```python
from build123d import *

# Parameters (mm, degrees)
SKETCH_1_W          = 350
SKETCH_1_H          = 140
EXTRUDE_1_DEPTH     = 1.5
SKETCH_2_W          = 220
SKETCH_2_H          = 110
CUT_EXTRUDE_1_DEPTH = 2
EXTRUDE_1_2_DEPTH   = 15
SKETCH_4_W          = 221.5
SKETCH_4_H          = 1.5
EXTRUDE_3_DEPTH     = 100
FILLET_1_R          = 10
CUT_EXTRUDE_2_DEPTH = 100


with BuildPart() as part:
    # 草图1 → Extrude 1 (new body)
    with BuildSketch(Plane.XY):
        Rectangle(SKETCH_1_W, SKETCH_1_H)
    extrude(amount=EXTRUDE_1_DEPTH)

    # 草图2 → 切除-拉伸1 (cut)
    with BuildSketch(Plane.XY.offset(1.5)):
        with Locations((65, 15)):
            Rectangle(SKETCH_2_W, SKETCH_2_H)
    extrude(amount=-CUT_EXTRUDE_1_DEPTH, mode=Mode.SUBTRACT)

    # 草图3 → Extrude 1 2 (add)
    with BuildSketch(Plane.XY.offset(1.5)):
        Polygon((175, -40), (175, -70), (-175, -70), (-175, 70), (-45, 70), (-45, -40), (-46.5, -40), (-46.5, 68.5), (-173.5, 68.5), (-173.5, -68.5), (173.5, -68.5), (173.5, -40), align=None)
    extrude(amount=EXTRUDE_1_2_DEPTH)

    # 草图4 → 凸台-拉伸3 (add)
    with BuildSketch(Plane.XY.offset(1.5)):
        with Locations((64.25, -40.75)):
            Rectangle(SKETCH_4_W, SKETCH_4_H)
    extrude(amount=EXTRUDE_3_DEPTH)

    # 圆角1
    fillet_1_edges = [part.edges().sort_by_distance(p)[0] for p in [
        (-46.5, -40.75, 101.5),
        (175, -40.75, 101.5),
    ]]
    fillet(fillet_1_edges, radius=FILLET_1_R)

    # 草图5 → 切除-拉伸2 (cut)
    with BuildSketch(Plane.XZ.offset(41.5)):
        with BuildLine():
            Line((-18, 82.5), (-18, 57.5))
            ThreePointArc((-18, 57.5), (-24, 51.5), (-30, 57.5))
            Line((-30, 57.5), (-30, 82.5))
            ThreePointArc((-30, 82.5), (-24, 88.5), (-18, 82.5))
        make_face()
        with BuildLine():
            Line((164, 82.5), (164, 57.5))
            ThreePointArc((164, 57.5), (158, 51.5), (152, 57.5))
            Line((152, 57.5), (152, 82.5))
            ThreePointArc((152, 82.5), (158, 88.5), (164, 82.5))
        make_face()
    extrude(amount=-CUT_EXTRUDE_2_DEPTH, mode=Mode.SUBTRACT)


solid = part.part
```
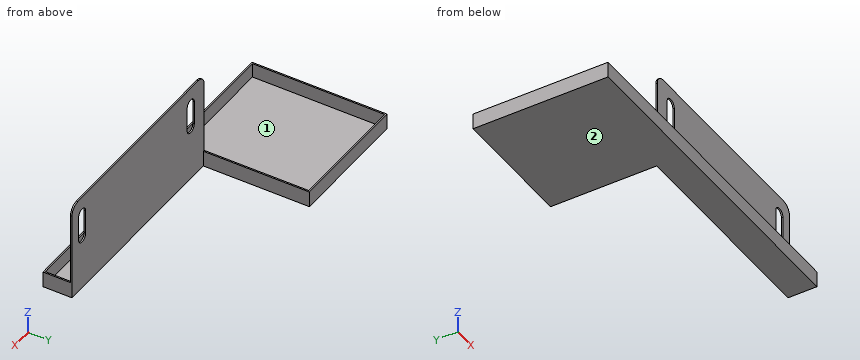
The listing builds one solid part. Answer for the finished solid, in the listing's coordinates (mm). Face numbers are marked on the shaded views. Coordinates: 2 decimals unless noted, no trailing zeros. Write each loop counter-clockwise with the first axis right and the second up, starting at its lowest first coordinate (ties: lowest second). Pieces come first, ordered by that corner, then holes. Notation, with made-up numbers: (75.25, -5.5) - (123.25, -5.5) arc R29 ccw to (123.25, 30.5) - close; hole circle Ø5 at (30.25, 35.25). An arc over 180 degrees is marked (long way). Return JSON: item names as keys, results as strings. Group by question number.
1. A cutting plane is placed at B-B, the plane z = 73. Determine the outline of the cut face in (x, y), plus the area to 3 significant figures.
2. Straight lines are drawn through the part: L1, parallel to Y at x = 58, z = 11.5; L2, parallel to Y at x = -7, z = 78; L3, parallel to Z at x = -49, y = 31. For each, find the intervals that lie inside material, in ascending order.
3. Given pin 1 (12 mm diameter, centred on x = 4.5, z = 29.5, fed in from -Y); pin 2 (16.5 mm diameter, centred on x = 35, z = 10, fed in from +Y); pin 3 (4.5 mm diameter, centred on y = 6.5, z = 10, fed in from +X), each flat-ended and moving along its own axis, determine where each tip first touches the part or whether it passes through.
4. A cutting plane is placed at C-C, the plane y = -49.5. Determine the outline of the cut face in (x, z).
5. Determine the mould class of the marked faces 1 and 2 for opening direction Y: released by +Y, released by -Y, zero draft, split by the parting line, or undercut.
6. A cutting plane is placed at D-D, the plane x = -60. Determine the outline of the cut face in (y, z).
7. A cutting plane is placed at A-A, the plane x = 158. Determine the outline of the cut face in (y, z), plus the area to 3 significant figures.
Ans:
{
 "1": {"outline": "(-46.5, -41.5) - (-30, -41.5) - (-30, -40) - (-46.5, -40) - close; (-18, -41.5) - (152, -41.5) - (152, -40) - (-18, -40) - close; (164, -41.5) - (175, -41.5) - (175, -40) - (164, -40) - close", "area": "296 mm²"},
 "2": {"L1": "-70 to -68.5, -41.5 to -40", "L2": "-41.5 to -40", "L3": "0 to 1.5"},
 "3": {"pin 1": "y = -41.5", "pin 2": "y = -40", "pin 3": "x = -45"},
 "4": {"outline": "(-175, 0) - (175, 0) - (175, 16.5) - (173.5, 16.5) - (173.5, 1.5) - (-173.5, 1.5) - (-173.5, 16.5) - (-175, 16.5) - close"},
 "5": {"face 1": "undercut", "face 2": "zero draft"},
 "6": {"outline": "(-70, 0) - (70, 0) - (70, 16.5) - (68.5, 16.5) - (68.5, 1.5) - (-68.5, 1.5) - (-68.5, 16.5) - (-70, 16.5) - close"},
 "7": {"outline": "(-70, 0) - (-40, 0) - (-40, 51.5) - (-41.5, 51.5) - (-41.5, 1.5) - (-68.5, 1.5) - (-68.5, 16.5) - (-70, 16.5) - close; (-41.5, 88.5) - (-40, 88.5) - (-40, 101.5) - (-41.5, 101.5) - close", "area": "162 mm²"}
}
